```python
from build123d import *

# Parameters (mm, degrees)
SKETCH1_W                                         = 600
SKETCH1_H                                         = 160
EXTRUDE1_DEPTH                                    = 6
M6_SOCKET_HEAD_CAP_SCREW_COUNTERBORE1_D           = 6.6
M6_SOCKET_HEAD_CAP_SCREW_COUNTERBORE1_CBORE_D     = 11
M6_SOCKET_HEAD_CAP_SCREW_COUNTERBORE1_CBORE_DEPTH = 7
M4_TAPPED_HOLE1_D                                 = 3.3
M4_TAPPED_HOLE1_DEPTH                             = 10.1
M4_TAPPED_HOLE1_TIP                               = 0.991420021
M8_TAPPED_HOLE1_D                                 = 6.8
M6_TAPPED_HOLE2_D                                 = 5
SKETCH10_R                                        = 20
CUT_EXTRUDE1_DEPTH                                = 311.715303775
M4_TAPPED_HOLE2_D                                 = 3.3
M4_TAPPED_HOLE2_DEPTH                             = 12
M4_TAPPED_HOLE2_TIP                               = 0.991420021
CHAMFER1_SIZE                                     = 5
SKETCH13_R                                        = 5
CUT_EXTRUDE2_DEPTH                                = 311.715303775


with BuildPart() as part:
    # Sketch1 → Extrude1 (new, symmetric)
    with BuildSketch(Plane(origin=(0, 0, 0), x_dir=(1, 0, 0), z_dir=(0, 1, 0))):
        Rectangle(SKETCH1_W, SKETCH1_H)
    extrude(amount=EXTRUDE1_DEPTH, both=True)

    # M6 Socket Head Cap Screw Counterbore1 (through all)
    with Locations(Plane(origin=(-280, 6, 60), x_dir=(0, 0, 1), z_dir=(0, 1, 0))):
        with Locations((0, 0), (-100, 0), (0, 480), (-115, 480), (-115, 560), (0, 560)):
            CounterBoreHole(M6_SOCKET_HEAD_CAP_SCREW_COUNTERBORE1_D / 2, M6_SOCKET_HEAD_CAP_SCREW_COUNTERBORE1_CBORE_D / 2, M6_SOCKET_HEAD_CAP_SCREW_COUNTERBORE1_CBORE_DEPTH)

    # M4 Tapped Hole1
    with Locations(Plane(origin=(270, 0, -80), x_dir=(-1, 0, 0), z_dir=(0, 0, -1))):
        with Locations((0, 0), (250, 0), (500, 0)):
            Hole(M4_TAPPED_HOLE1_D / 2, depth=M4_TAPPED_HOLE1_DEPTH)
            with Locations((0, 0, -(M4_TAPPED_HOLE1_DEPTH + M4_TAPPED_HOLE1_TIP / 2))):  # 118° drill point
                Cone(0, M4_TAPPED_HOLE1_D / 2, M4_TAPPED_HOLE1_TIP, mode=Mode.SUBTRACT)

    # M8 Tapped Hole1 (through all)
    with Locations(Plane(origin=(-174, 6, 19), x_dir=(0, 0, 1), z_dir=(0, 1, 0))):
        with Locations((0, 0), (0, 50), (-55, 50), (-55, 0)):
            Hole(M8_TAPPED_HOLE1_D / 2)

    # M6 Tapped Hole2 (through all)
    with Locations(Plane(origin=(55, 6, 60), x_dir=(0, 0, 1), z_dir=(0, 1, 0))):
        with Locations((0, 0), (0, -250)):
            Hole(M6_TAPPED_HOLE2_D / 2)

    # Sketch10 → Cut-Extrude1 (cut, through all)
    with BuildSketch(Plane(origin=(0, 6, 0), x_dir=(1, 0, 0), z_dir=(0, 1, 0))):
        with Locations(Location((-230, 10, 0), (0, 0, 270))):
            Circle(SKETCH10_R)
    extrude(amount=-CUT_EXTRUDE1_DEPTH, mode=Mode.SUBTRACT)

    # M4 Tapped Hole2
    with Locations(Plane(origin=(-25, 6, -5), x_dir=(0, 0, 1), z_dir=(0, 1, 0))):
        with Locations((0, 0), (-25, 0)):
            Hole(M4_TAPPED_HOLE2_D / 2, depth=M4_TAPPED_HOLE2_DEPTH)
            with Locations((0, 0, -(M4_TAPPED_HOLE2_DEPTH + M4_TAPPED_HOLE2_TIP / 2))):  # 118° drill point
                Cone(0, M4_TAPPED_HOLE2_D / 2, M4_TAPPED_HOLE2_TIP, mode=Mode.SUBTRACT)

    # Chamfer1
    chamfer1_edges = [part.edges().sort_by_distance(p)[0] for p in [
        (300, 0, 80),
        (-300, 0, 80),
    ]]
    chamfer(chamfer1_edges, length=CHAMFER1_SIZE)

    # Sketch13 → Cut-Extrude2 (cut, through all)
    with BuildSketch(Plane(origin=(0, 6, 0), x_dir=(1, 0, 0), z_dir=(0, 1, 0))):
        with Locations(Location((-45, 17.5, 0), (0, 0, 270))):
            Circle(SKETCH13_R)
    extrude(amount=-CUT_EXTRUDE2_DEPTH, mode=Mode.SUBTRACT)


solid = part.part
```
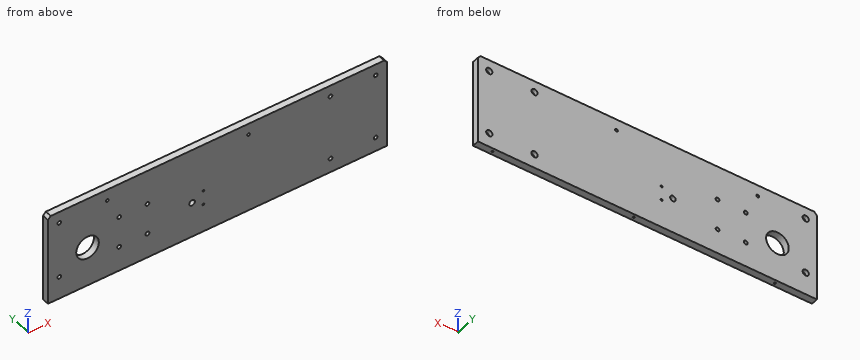
The listing builds one solid part. Answer for the finished solid, in the listing's coordinates (mm). Coordinates: 2 decimals unless noted, no trailing zeros. Write each loop counter-clockwise with the first axis right and the second up, starting at its lowest first coordinate (ties: lowest second). Pieces come first, ordered by that corner, then holes. Notation, with made-up numbers: (57.25, 84.5) -> (81.25, 84.5) arc R16 ccw to (81.25, 101.5) -> close; hole circle Ø7 at (72, 39.25). An arc over 180 degrees is marked (long way). Write each question's results on one line, items separated by ' | '. Start each with the question number.
1) A cutting plane is placed at A-A (x = -45). Determine the outline of the cut face in (y, z), then the cut area to 3 significant figures.
2) Flat-ended cylindrical pins translate along their axes: pin 1 Ø5.5 at (x, z) = (-25, -30) entering from -Y; pin 2 Ø9 at (x, z) = (200, -55) entering from +Y. Find the tip coordinate at first contact, or state that the pin passes through.
3) Straight lines are drawn through the part: probe 1 along X at (y, z) = (-4.25, -55); probe 2 along X at (y, z) = (-2.75, 60); probe 3 along Z at (x, y) = (-280, 2.5). For each, find the intervals that lie inside material, in ascending order.
Values follow:
1) outline: (-6, -80) -> (6, -80) -> (6, -22.5) -> (-6, -22.5) -> close; (-6, -12.5) -> (6, -12.5) -> (6, 80) -> (-6, 80) -> close | area: 1,800 mm²
2) pin 1: y = -6 | pin 2: y = -1
3) probe 1: -300 to 196.7, 203.3 to 276.7, 283.3 to 300 | probe 2: -300 to -283.3, -276.7 to -197.5, -192.5 to 52.5, 57.5 to 196.7, 203.3 to 276.7, 283.3 to 300 | probe 3: -80 to -45.5, -34.5 to 54.5, 65.5 to 80
